Design review of the part built by this model. Coordinates are the model's own, in mm. Face numbers are marked on the shaded views. A direction names the side the tool comes from. Give positions to 0.01 mm unless a question says otherwise; leave off trailing zeros. Order: outer loops, then holes, each group sorted by start corner. A loop starts at its lowest first (then second) coordinate and runs counter-clockwise, first axis right, second up. Notation, with made-up numbers: M 88.25,66 L 147.25,66 A8 cw 147.25,70 Z; hole C -17.75,-39.5 d7. An arc over 180 degrees is marked long. Put each result on its own line as item: value. Start each with the question number.
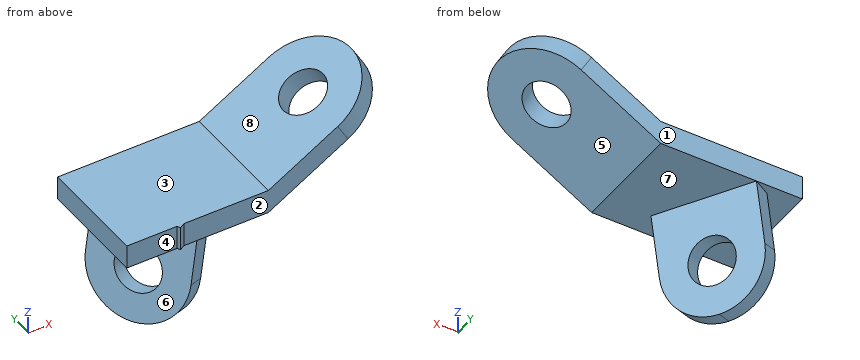
from build123d import *

# Parameters (mm, degrees)
BASE_PLATE_SKETCH_W         = 77
BASE_PLATE_SKETCH_H         = 60
BASE_PLATE_60X77X13_DEPTH   = 13
UPPER_EYE_LUG_DEPTH         = 30
UPPER_LUG_CUT_SKETCH_R      = 12.5
UPPER_LUG_CUT_DEPTH         = 13
LOWER_EYE_LUG_DEPTH         = 13
LOWER_EYE_LUG_DEPTH_BACK    = 62
LOWER_LUG_PROFILE_CUT_DEPTH = 62
LOWER_LUG_TRIM_SKETCH_R     = 12.5
LOWER_LUG_TRIM_CUT_DEPTH    = 62


with BuildPart() as part:
    # Base Plate Sketch → Base Plate 60x77x13 (new body)
    with BuildSketch(Plane.XY):
        Rectangle(BASE_PLATE_SKETCH_W, BASE_PLATE_SKETCH_H)
    extrude(amount=BASE_PLATE_60X77X13_DEPTH)

    # Upper Lug Sketch → Upper Eye Lug (add, symmetric)
    with BuildSketch(Plane(origin=(0, 0, 0), x_dir=(1, 0, 0), z_dir=(0, 1, 0))):
        Polygon((38.5, -13), (38.5, 0), (120.77241336, -47.5), (112.112159322, -55.5), align=None)
    extrude(amount=UPPER_EYE_LUG_DEPTH, both=True)

    # Upper Lug Cut Sketch → Upper Lug Cut (cut)
    with BuildSketch(Plane(origin=(9.625, 0, -16.670989023), x_dir=(-0.8660254037844419, 0, -0.49999999999999434), z_dir=(0.49999999999999434, 0, -0.8660254037844419))):
        with BuildLine():
            Line((-128.341978046, 30), (-128.341978046, -30))
            Line((-128.341978046, -30), (-83.341978046, -30))
            ThreePointArc((-83.341978046, -30), (-113.341978046, 0), (-83.341978046, 30))
            Line((-83.341978046, 30), (-128.341978046, 30))
        make_face()
        with Locations((-83.341978046, 0)):
            Circle(UPPER_LUG_CUT_SKETCH_R)
    extrude(amount=-UPPER_LUG_CUT_DEPTH, mode=Mode.SUBTRACT)

    # Lower Lug Sketch → Lower Eye Lug (add, two sides: drawn at the far end of the back side and taken through both)
    with BuildSketch(Plane.XY.offset(-LOWER_EYE_LUG_DEPTH_BACK)):
        Polygon((14, -17.631397208), (-10.248711306, -31.631397208), (-37.748711306, 16), (-13.5, 30), align=None)
    extrude(amount=LOWER_EYE_LUG_DEPTH + LOWER_EYE_LUG_DEPTH_BACK)

    # Lower Lug Profile Cut Sketch → Lower Lug Profile Cut (cut)
    with BuildSketch(Plane(origin=(-16.365381057, 28.345671476, 0), x_dir=(0.8660254037844398, 0.4999999999999981, 0), z_dir=(-0.49999999999999817, 0.8660254037844398, 0))):
        Polygon((-7.044104755, 0), (-22.768294497, 60), (-12.768294497, 60), (3.308657049, 0), (3.308657049, 62), (-24.691342951, 62), (-24.691342951, 0), align=None)
    extrude(amount=-LOWER_LUG_PROFILE_CUT_DEPTH, mode=Mode.SUBTRACT)

    # Lower Lug Trim Sketch → Lower Lug Trim Cut (cut)
    with BuildSketch(Plane(origin=(2.673436922, 1.543509526, -0.827164262), x_dir=(-0.22414386804201733, -0.129409522551262, -0.9659258262890672), z_dir=(0.836516303737808, 0.48296291314453194, -0.258819045102525))):
        with BuildLine():
            Line((31.143656542, -22.269237886), (61.260227367, -22.269237886))
            Line((61.260227367, -22.269237886), (61.260227367, 32.730762114))
            Line((61.260227367, 32.730762114), (31.143656542, 32.730762114))
            ThreePointArc((31.143656542, 32.730762114), (50.589093025, 24.676198596), (58.643656542, 5.230762114))
            ThreePointArc((58.643656542, 5.230762114), (50.589093025, -14.214674369), (31.143656542, -22.269237886))
        make_face()
        with Locations(Location((31.143656542, 5.230762114, 0), (0, 0, 90))):
            Circle(LOWER_LUG_TRIM_SKETCH_R)
    extrude(amount=-LOWER_LUG_TRIM_CUT_DEPTH, mode=Mode.SUBTRACT)


with BuildPart() as body_2:
    # of the pieces the cut leaves, the one that is kept (lower_lug_trim_cut_keep)
    add(part.part.solids().sort_by_distance((-38.5, 30, 0))[0])


solid = body_2.part
1. Consider section B-B on z = -9. Give the boundary of the cut face in (x, y), then the cut area to 3 significant figures.
2. To check wall thickness, follow probe 1 along Z at (x, y) = (13, -27.5); probe 2 along Y at (x, z) = (90.5, 33); probe 3 along Y at (x, z) = (-27.5, -48). State the ranges of each line that lie inside material, in increasing order.
3. Consider section A-A on x = 21. Give the boundary of the cut face in (y, z).
4. The part is to be moulded in two halves that separate along Z. For the marked faces 5, 6, 7 and 8, say which applies: +Z half, -Z half, draft (parallel to the pull), parting line (faces both ways), or undercut.
5. Machinability: for the marked faces 1, 2, 3 and 4, which of the approach directions +Z, -Z, +X, -X, +Y, -Y give a long, thin tool a straight path to every point of the face, cutting with its end or side? Answer none if there is none.
6. Insertion check: pin 1 (12 mm diameter, centred on x = 54, y = 22, fed in from -Z); pin 2 (17.5 mm diameter, centred on x = 29.5, z = 15.5, fed in from -Y); pin 3 (1 mm diameter, centred on y = 17, z = -18, fed in from -X); pin 4 (5 mm diameter, centred on x = 40, z = 19.5, fed in from -Y). Each pin has a flat end and moves straight along its axis. Give the tip position at first contact, or say it passes through.
7. Consider section C-C on y = 6. Give the number of separate pieces and of enclosed holes in the cut face, then the cut area to 3 significant figures.
Returned:
1. outline: M -24.51,23.64 L 2.99,-23.99 L 11.91,-18.84 L -15.59,28.79 Z
1. area: 566 mm2
2. probe 1: z = 0 to 13
2. probe 2: y = -27.69 to -4.82, 4.82 to 27.69
2. probe 3: y = 8.38 to 12.19
3. outline: M -30,0 L 30,0 L 30,13 L -30,13 Z
4. face 5: -Z half
4. face 6: undercut
4. face 7: undercut
4. face 8: +Z half
5. face 1: +Z, -Z, +X, -X, +Y
5. face 2: +Z, -Z, +X, -Y
5. face 3: +Z, -X, +Y, -Y
5. face 4: +Z, -Z, -X, -Y
6. pin 1: stops at z = 5.48
6. pin 2: stops at y = -30
6. pin 3: stops at x = -23.72
6. pin 4: passes through
7. separate pieces: 3
7. enclosed holes: 0
7. area: 2,020 mm2
